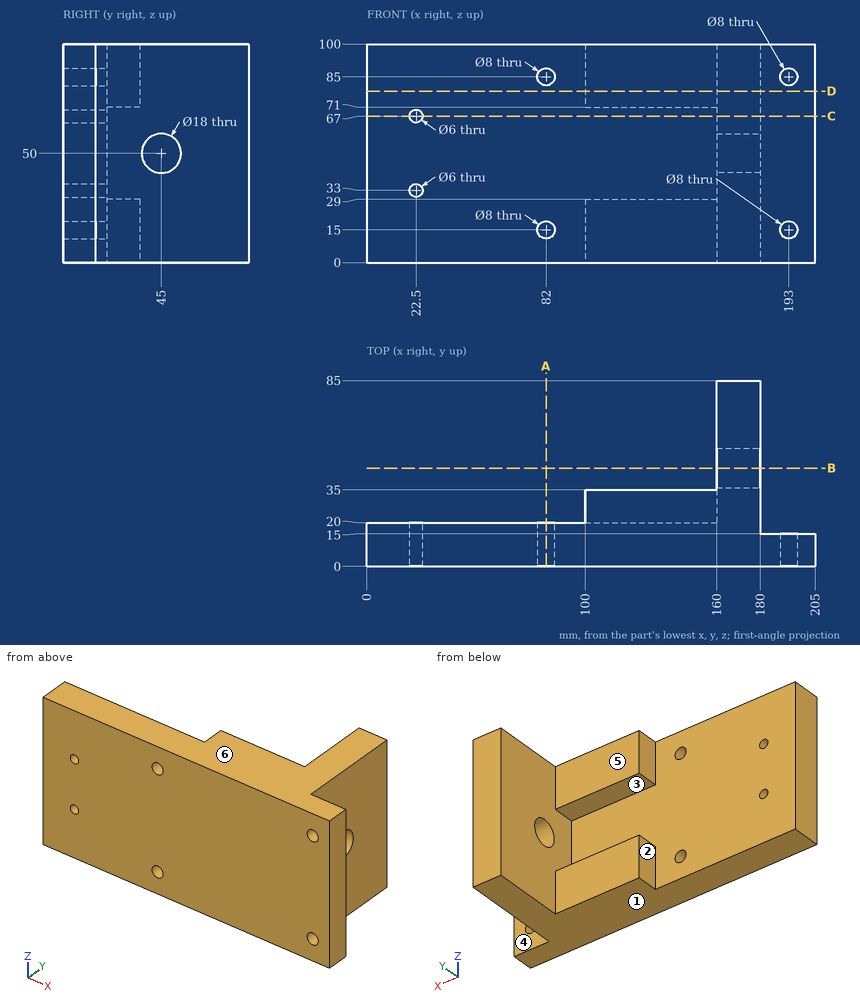
Geometry check sheet. Reference: drawing and pictorial views, mm from the part's lowest x, y, z. A direction names the side the tool comes from. Round coordinates to 2 decimals unless told otherwise and drop trailing zeros. Loops run counter-clockwise (first coordinate to the right, second up) from the corner with the lowest first, then second, coordinate; pieces in that order, holes last. Notation, with made-up numbers: (70.5, 35.25) -> (108.5, 35.25) arc R10 ccw to (108.5, 50.25) -> close; hole circle Ø2 at (63, 9). An arc over 180 degrees is marked (long way). Use a Markdown table: item, result.
(1) Go/stop test with flat-tipped pins: P1, Ø6, axis at x = 184, y = 65, coming from the +Z side; P2, Ø20.5, axis at y = 45, z = 50, coming from the -X side; P3, Ø10.5, axis at x = 193, z = 85, coming from the +Y side; P4, Ø8.5, axis at x = 132.5, z = 14, coming from the +Y side. Record where each tip stops, or that it passes through.
Calculated:
| item | result |
|---|---|
| P1 | through |
| P2 | x = 160 |
| P3 | y = 15 |
| P4 | y = 35 |
(2) Sectioned sample at D-D (z = 78.5). Enter the section's corners in (x, y).
Calculated:
| item | result |
|---|---|
| outline | (0, 0) -> (205, 0) -> (205, 15) -> (180, 15) -> (180, 85) -> (160, 85) -> (160, 35) -> (100, 35) -> (100, 20) -> (0, 20) -> close |
(3) Sectioned sample at C-C (z = 67). Enter the section's corners in (x, y).
Calculated:
| item | result |
|---|---|
| outline | (0, 0) -> (19.5, 0) -> (19.5, 20) -> (0, 20) -> close; (25.5, 0) -> (205, 0) -> (205, 15) -> (180, 15) -> (180, 85) -> (160, 85) -> (160, 20) -> (25.5, 20) -> close |
(4) Set-up check for the marked faces 4, 5 and 6: record each of +Z, -Z, +X, -X, +Y, -Y from which the full face is reachable in a straight line by a thin tool's end or side.
Calculated:
| item | result |
|---|---|
| face 4 | +Z, -Z, +X, +Y |
| face 5 | +Z, -Z, -X, +Y |
| face 6 | +Z, +X, -X, +Y, -Y |
(5) Sectioned sample at A-A (x = 82). Enter the section's corners in (y, z), then the cut area to 3 significant figures.
Calculated:
| item | result |
|---|---|
| outline | (0, 0) -> (20, 0) -> (20, 11) -> (0, 11) -> close; (0, 19) -> (20, 19) -> (20, 81) -> (0, 81) -> close; (0, 89) -> (20, 89) -> (20, 100) -> (0, 100) -> close |
| area | 1,680 mm² |
(6) Sectioned sample at B-B (y = 45). Enter the section's corners in (x, z), then the cut area to 3 significant figures.
Calculated:
| item | result |
|---|---|
| outline | (160, 0) -> (180, 0) -> (180, 41) -> (160, 41) -> close; (160, 59) -> (180, 59) -> (180, 100) -> (160, 100) -> close |
| area | 1,640 mm² |
(7) Mould release check, pull along Z, two halves, no side actions. Record for the marked faces 1, 2 and 3: released by +Z, released by -Z, zero draft, split by the parting line, or undercut.
Calculated:
| item | result |
|---|---|
| face 1 | released by -Z |
| face 2 | zero draft |
| face 3 | undercut |
(8) Scan lines: probe 1 along Z at (x, y) = (22, 9); probe 2 along Z at (x, y) = (82, 14); probe 3 along Z at (x, y) = (121.5, 30.5). Record each from-to range of solid material in increasing order.
Calculated:
| item | result |
|---|---|
| probe 1 | 0 to 30.04, 35.96 to 64.04, 69.96 to 100 |
| probe 2 | 0 to 11, 19 to 81, 89 to 100 |
| probe 3 | 0 to 29, 71 to 100 |
